```python
from build123d import *

# Parameters (mm, degrees)
BOSS_EXTRUDE1_DEPTH = 70
SKETCH2_R           = 20
CUT_EXTRUDE1_DEPTH  = 10
SKETCH3_R           = 27.5
BOSS_EXTRUDE2_DEPTH = 10
SKETCH4_R           = 17.5
BOSS_EXTRUDE3_DEPTH = 30


with BuildPart() as part:
    # Sketch1 → Boss-Extrude1 (new body)
    with BuildSketch(Plane(origin=(0, 0, 0), x_dir=(1, 0, 0), z_dir=(0, 1, 0))):
        with BuildLine():
            Line((5, 35), (35, 35))
            Line((35, 35), (35, 5))
            ThreePointArc((35, 5), (30, 0), (35, -5))
            Line((35, -5), (35, -35))
            Line((35, -35), (5, -35))
            ThreePointArc((5, -35), (0, -30), (-5, -35))
            Line((-5, -35), (-35, -35))
            Line((-35, -35), (-35, -5))
            ThreePointArc((-35, -5), (-30, 0), (-35, 5))
            Line((-35, 5), (-35, 35))
            Line((-35, 35), (-5, 35))
            ThreePointArc((-5, 35), (0, 30), (5, 35))
        make_face()
    extrude(amount=BOSS_EXTRUDE1_DEPTH)

    # Sketch2 → Cut-Extrude1 (cut)
    with BuildSketch(Plane.XZ):
        with Locations(Location((0, 0, 0), (0, 0, 270))):
            Circle(SKETCH2_R)
    extrude(amount=-CUT_EXTRUDE1_DEPTH, mode=Mode.SUBTRACT)

    # Sketch3 → Boss-Extrude2 (add)
    with BuildSketch(Plane(origin=(0, 70, 0), x_dir=(1, 0, 0), z_dir=(0, 1, 0))):
        with Locations(Location((0, 0, 0), (0, 0, 270))):
            Circle(SKETCH3_R)
    extrude(amount=BOSS_EXTRUDE2_DEPTH)

    # Sketch4 → Boss-Extrude3 (add)
    with BuildSketch(Plane(origin=(0, 80, 0), x_dir=(1, 0, 0), z_dir=(0, 1, 0))):
        with Locations(Location((0, 0, 0), (0, 0, 270))):
            Circle(SKETCH4_R)
    extrude(amount=BOSS_EXTRUDE3_DEPTH)


solid = part.part
```
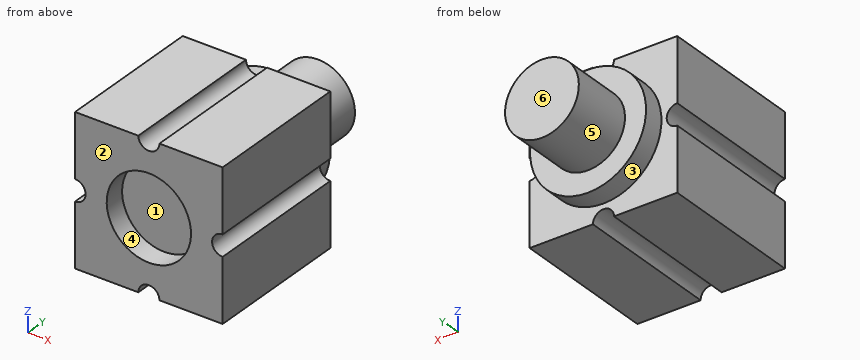
CAD build for the part. Positions are in the model's coordinates, mm. Face numbers are marked on the shaded views. A direction names the side the tool comes from. Give positions to 0.01 mm unless a question says otherwise; leave off trailing zeros. Order: outer loops, then holes, each group sorted by start corner. A loop starts at its lowest first (then second) coordinate and runs counter-clockwise, first axis right, second up. Notation, with made-up numbers: M 29.25,69.5 L 45.25,69.5 A14 ccw 45.25,73.5 Z; hole C 60,69.5 d11. An arc over 180 degrees is marked long. Put each result on its own line as item: value. Start each with the question number.
(1) Saw through at C-C, the plane x = 0. Write the cut outline in (y, z), then the cut area to 3 significant figures.
(2) Saw through at B-B, the plane y = 66.5. Write the cut outline in (x, z), then the cut area to 3 significant figures.
(3) Which spindle directions (+Z, -Z, +X, -X, +Y, -Y) get a long thin tool onto all of the face, cutting with end or side? Do the marked faces 1, 2 and 3. Say none if no direction does.
(4) Drill centre lines: line 1 along X through (y, z) = (3, 0); line 2 along Y through (x, z) = (25, -6); line 3 along Y through (x, z) = (-28, 11). Where is each one in solid material? Low to high.
(5) Saw through at A-A, the plane z = 0. Write the cut outline in (x, y).
(6) Flat gauge pins, fed straight in: pin 1 Ø12 at (x, z) = (-3.5, 4) entering from -Y; pin 2 Ø2 at (y, z) = (83.5, -14) entering from -X; pin 3 Ø1.5 at (x, z) = (-22.5, -22.5) entering from +Y. Where does each tip first touch, or does it go through?
(7) Saw through at D-D, the plane z = 22.5. Write the cut outline in (x, y).
(8) Mould opens along X. For the marked faces 4, 5 and 6 say: +X half, -X half, draft (parallel to the pull), parting line (faces both ways), or undercut.
Check result:
1. outline: M 0,-30 L 70,-30 L 70,-27.5 L 80,-27.5 L 80,-17.5 L 110,-17.5 L 110,17.5 L 80,17.5 L 80,27.5 L 70,27.5 L 70,30 L 0,30 L 0,20 L 10,20 L 10,-20 L 0,-20 Z
1. area: 5,400 mm2
2. outline: M -35,-35 L -5,-35 A5 cw 5,-35 L 35,-35 L 35,-5 A5 cw 35,5 L 35,35 L 5,35 A5 cw -5,35 L -35,35 L -35,5 A5 cw -35,-5 Z
2. area: 4,740 mm2
3. face 1: -Y
3. face 2: +Z, -Z, +X, -X, -Y
3. face 3: +Y
4. line 1: x = -30 to -20, 20 to 30
4. line 2: y = 0 to 80
4. line 3: y = 0 to 70
5. outline: M -30,0 L -20,0 L -20,10 L 20,10 L 20,0 L 30,0 L 30,70 L 27.5,70 L 27.5,80 L 17.5,80 L 17.5,110 L -17.5,110 L -17.5,80 L -27.5,80 L -27.5,70 L -30,70 Z
6. pin 1: stops at y = 10
6. pin 2: stops at x = -11.72
6. pin 3: stops at y = 70
7. outline: M -35,0 L 35,0 L 35,70 L 15.81,70 L 15.81,80 L -15.81,80 L -15.81,70 L -35,70 Z
8. face 4: undercut
8. face 5: parting line
8. face 6: draft
